Geometry: final body of the model. Coordinates: model frame, mm. A direction names the side the tool comes from. Coordinates: 2 decimals unless noted, no trailing zeros. Write each loop counter-clockwise with the first axis right and the second up, starting at its lowest first coordinate (ties: lowest second). Pieces come first, ordered by that corner, then holes. Notation, with made-up numbers: M -9.75,28.5 L -5.75,28.5 A17 ccw -5.75,33.5 Z; hole C -1,53.25 d4. An arc over 180 degrees is marked long. Write item = value, one per line. Start each with the question number.
Item 1: First-contact query: pin 1 Ø3 at (x, z) = (72, 7) entering from -Y; pin 2 Ø1.5 at (y, z) = (-39.5, 41) entering from +X; pin 3 Ø8 at (y, z) = (-114, 33.5) entering from -X. Flat tips, straight axial feed; report the tip coordinate or a pass-through.
Item 2: Section B-B on y = -20. Output: boundary loops of the cut face in (x, z), plus the area to 3 significant figures.
Item 3: Section D-D on y = -88. Output: boundary loops of the cut face in (x, z), plus the area to 3 significant figures.
Item 4: Section C-C on x = 82.5. Output: boundary loops of the cut face in (y, z).
Item 5: Ray query, L1, parallel to Y at x = 68.5, z = 19; L2, parallel to X at y = -90, z = 9; L3, parallel to Y at x = -3.25, z = 30. Return the intervals inside material, ascending. Write a range as [from, to].
Item 6: Section A-A on z = 30. Output: boundary loops of the cut face in (x, y).
Item 7: Reachability of faces 1 (the flat face through (-2.465, -43.552, 52.984)), 2 (the flat face through (95, -117, 30)), 3 (the flat face through (97, -117, 45.5)) from +Z, -Z, +X, -X, +Y, -Y: full face, straight path, thin tool, end or side. Return the list, or none.
Item 8: Pull-direction query (Y, two-part tool) for faces 4 (the flat face through (98, -118, 5.5)), 5 (the flat face through (51, -99, 0)), 6 (the flat face through (47, -95, 30)), 7 (the flat face through (48, -100, 30)); classes: +Y half, -Y half, draft (parallel to the pull), parting line (faces both ways), or undercut.
from build123d import *

# Parameters (mm, degrees)
BOSS_EXTRUDE1_DEPTH            = 5
SKETCH2_W                      = 60
SKETCH2_H                      = 35
BOSS_EXTRUDE2_DEPTH            = 100
SKETCH3_W                      = 100
SKETCH3_H                      = 30
CUT_EXTRUDE1_DEPTH             = 175.642491966
CUT_EXTRUDE2_DEPTH             = 175.642491966
CUT_EXTRUDE3_DEPTH             = 178.552809046
F_18_0_18_DIAMETER_HOLE1_D     = 18
F_18_0_18_DIAMETER_HOLE1_DEPTH = 105
FILLET1_R                      = 3
FILLET2_R                      = 8
FILLET3_R                      = 10


with BuildPart() as part:
    # Sketch1 → Boss-Extrude1 (new body)
    with BuildSketch(Plane(origin=(0, 0, 0), x_dir=(0, 0, -1), z_dir=(1, 0, 0))):
        Polygon((0, -80), (-14.600649986, 0), (-44.600649986, 0), (-60, -80), (-60, -130), (0, -130), align=None)
    extrude(amount=-BOSS_EXTRUDE1_DEPTH)

    # Sketch2 → Boss-Extrude2 (add)
    with BuildSketch(Plane(origin=(0, 0, 0), x_dir=(0, 0, -1), z_dir=(1, 0, 0))):
        with Locations((-30, -112.5)):
            Rectangle(SKETCH2_W, SKETCH2_H)
    extrude(amount=BOSS_EXTRUDE2_DEPTH)

    # Sketch3 → Cut-Extrude1 (cut, through all)
    with BuildSketch(Plane(origin=(0, 0, 0), x_dir=(-1, 0, 0), z_dir=(0, 0, -1))):
        with Locations((-45, -115)):
            Rectangle(SKETCH3_W, SKETCH3_H)
    extrude(amount=-CUT_EXTRUDE1_DEPTH, mode=Mode.SUBTRACT)

    # Sketch4 → Cut-Extrude2 (cut, through all)
    with BuildSketch(Plane.ZY.offset(-95)):
        with BuildLine():
            Line((54.5, -120.5), (54.5, -114.5))
            ThreePointArc((54.5, -114.5), (50, -110), (45.5, -114.5))
            Line((45.5, -114.5), (45.5, -120.5))
            ThreePointArc((45.5, -120.5), (50, -125), (54.5, -120.5))
        make_face()
    extrude(amount=-CUT_EXTRUDE2_DEPTH, mode=Mode.SUBTRACT)

    # Sketch5 → Cut-Extrude3 (cut, through all)
    with BuildSketch(Plane(origin=(100, 0, 0), x_dir=(0, 0, -1), z_dir=(1, 0, 0))):
        with BuildLine():
            Line((-14.5, -114.5), (-14.5, -120.5))
            ThreePointArc((-14.5, -120.5), (-10, -125), (-5.5, -120.5))
            Line((-5.5, -120.5), (-5.5, -114.5))
            ThreePointArc((-5.5, -114.5), (-10, -110), (-14.5, -114.5))
        make_face()
    extrude(amount=-CUT_EXTRUDE3_DEPTH, mode=Mode.SUBTRACT)

    # Ø18.0 (18) Diameter Hole1
    with Locations(Plane.ZY.offset(5)):
        with Locations((30, -20)):
            Hole(F_18_0_18_DIAMETER_HOLE1_D / 2, depth=F_18_0_18_DIAMETER_HOLE1_DEPTH)

    # Fillet1
    fillet1_edges = [part.edges().sort_by_distance(p)[0] for p in [
        (0, -95, 30),
        (95, -100, 30),
    ]]
    fillet(fillet1_edges, radius=FILLET1_R)

    # Fillet2
    fillet2_edges = [part.edges().sort_by_distance(p)[0] for p in [
        (100, -95, 30),
        (-5, -100, 30),
    ]]
    fillet(fillet2_edges, radius=FILLET2_R)

    # Fillet3
    fillet3_edges = [part.edges().sort_by_distance(p)[0] for p in [
        (-2.5, 0, 44.600649986),
        (-2.5, 0, 14.600649986),
        (97.5, -130, 60),
        (97.5, -130, 0),
    ]]
    fillet(fillet3_edges, radius=FILLET3_R)


solid = part.part
Responses:
q1.pin_1 = -100
q1.pin_2 = 0
q1.pin_3 = 95
q2.outline = M -5,10.95 L 0,10.95 L 0,21 L -5,21 Z; M -5,39 L 0,39 L 0,48.45 L -5,48.45 Z
q2.area = 97.5 mm²
q3.outline = M -5,0 L 0,0 L 0,60 L -5,60 Z
q3.area = 300 mm²
q4.outline = M -100,0 L -95,0 L -95,60 L -100,60 Z
q5.L1 = [-100, -95]
q5.L2 = [-5, 0]
q5.L3 = [-96.99, -29], [-11, 0]
q6.outline = M -5,-92 A8 ccw 3,-100 L 92,-100 A3 cw 95,-103 L 95,-130 L 100,-130 L 100,-103 A8 ccw 92,-95 L 3,-95 A3 cw 0,-92 L 0,-29 L -5,-29 Z; M -5,-11 L 0,-11 L 0,0 L -5,0 Z
q7.face_1 = +Z, +X, -X, +Y
q7.face_2 = +Z, -Z, -X, -Y
q7.face_3 = +X, -X
q8.face_4 = undercut
q8.face_5 = draft
q8.face_6 = +Y half
q8.face_7 = -Y half
